```python
from build123d import *

# Parameters (mm, degrees)
SKETCH_1_W          = 18
SKETCH_1_H          = 16
EXTRUDE_1_DEPTH     = 95
CHAMFER_1_SIZE      = 5
CUT_EXTRUDE_1_REACH = 100.005


with BuildPart() as part:
    # 草图1 → 凸台-拉伸1 (new, symmetric)
    with BuildSketch(Plane.XY):
        with Locations((9, 8)):
            Rectangle(SKETCH_1_W, SKETCH_1_H)
    extrude(amount=EXTRUDE_1_DEPTH, both=True)

    # 倒角1
    chamfer_1_edges = [part.edges().sort_by_distance(p)[0] for p in [
        (18, 8, -95),
        (18, 8, 95),
    ]]
    chamfer(chamfer_1_edges, length=CHAMFER_1_SIZE)

    # 草图2 → 切除-拉伸1 (cut, up to next)
    with BuildSketch(Plane.XZ, mode=Mode.PRIVATE) as cut_extrude_1_sk1:
        with BuildLine():
            Line((5.5, 83), (10.5, 83))
            ThreePointArc((10.5, 83), (13, 80.5), (10.5, 78))
            Line((10.5, 78), (5.5, 78))
            ThreePointArc((5.5, 78), (3, 80.5), (5.5, 83))
        make_face()
    cut_extrude_1_tool1 = extrude(cut_extrude_1_sk1.sketch, amount=-CUT_EXTRUDE_1_REACH, mode=Mode.PRIVATE) & part.part
    # 草图2 → 切除-拉伸1 (cut, up to next)
    with BuildSketch(Plane.XZ, mode=Mode.PRIVATE) as cut_extrude_1_sk2:
        with BuildLine():
            Line((5.5, 2.5), (10.5, 2.5))
            ThreePointArc((10.5, 2.5), (13, 0), (10.5, -2.5))
            Line((10.5, -2.5), (5.5, -2.5))
            ThreePointArc((5.5, -2.5), (3, 0), (5.5, 2.5))
        make_face()
    cut_extrude_1_tool2 = extrude(cut_extrude_1_sk2.sketch, amount=-CUT_EXTRUDE_1_REACH, mode=Mode.PRIVATE) & part.part
    # 草图2 → 切除-拉伸1 (cut, up to next)
    with BuildSketch(Plane.XZ, mode=Mode.PRIVATE) as cut_extrude_1_sk3:
        with BuildLine():
            Line((5.5, -83), (10.5, -83))
            ThreePointArc((10.5, -83), (13, -80.5), (10.5, -78))
            Line((10.5, -78), (5.5, -78))
            ThreePointArc((5.5, -78), (3, -80.5), (5.5, -83))
        make_face()
    cut_extrude_1_tool3 = extrude(cut_extrude_1_sk3.sketch, amount=-CUT_EXTRUDE_1_REACH, mode=Mode.PRIVATE) & part.part
    add(cut_extrude_1_tool1.solids().sort_by_distance((8, 0, 80.5))[0], mode=Mode.SUBTRACT)
    add(cut_extrude_1_tool2.solids().sort_by_distance((8, 0, 0))[0], mode=Mode.SUBTRACT)
    add(cut_extrude_1_tool3.solids().sort_by_distance((8, 0, -80.5))[0], mode=Mode.SUBTRACT)


solid = part.part
```
Work out the finished part from the listing and answer in its coordinate system (mm). A direction names the side the tool comes from. Give positions to 0.01 mm unless a question says otherwise; leave off trailing zeros. Order: outer loops, then holes, each group sorted by start corner. A loop starts at its lowest first (then second) coordinate and runs counter-clockwise, first axis right, second up. Notation, with made-up numbers: (68.5, -8) -> (72.5, -8) arc R30 cw to (72.5, 30) -> close; hole circle Ø3 at (62.25, -19.5). An arc over 180 degrees is marked (long way). Answer as CSV lines item,"result". Start each with the question number.
(1) Section A-A, the plane x = 7.25 is taken. Write down the section's boundary in (y, z).
(2) For a pull along X with two mould halves and no side action, classify faces 3 (the cylindrical face through (3, 8, 0)), 4 (the flat face through (8, 8, 2.5)), 5 (the flat face through (18, 8, 1)), 6 (the flat face through (6, 8, -95)) as released by +X, released by -X, zero draft, split by the parting line, or undercut.
(3) Section C-C, the plane z = -80.5 is taken. Write down the section's boundary in (x, y), plus the area to 3 significant figures.
(4) Consider line 1 along Z through (x, y) = (6.75, 12); line 2 along Z through (x, y) = (5, 13.5); line 3 along Z through (x, y) = (16.75, 3). Determine where each line is inside the solid, lowest interval first.
(5) Section B-B, the plane y = 12.5 is taken. Write down the section's boundary in (x, z).
(6) Which of the six approach directions +Z, -Z, +X, -X, +Y, -Y give full straight-line access (tool end or side, diameter ignored) to faces 1 (the flat face through (16, 8, 92)), 2 (the cylindrical face through (3, 7.9, -80.4))?
Entries:
1,outline,"(0, -95) -> (16, -95) -> (16, -83) -> (0, -83) -> close; (0, -78) -> (16, -78) -> (16, -2.5) -> (0, -2.5) -> close; (0, 2.5) -> (16, 2.5) -> (16, 78) -> (0, 78) -> close; (0, 83) -> (16, 83) -> (16, 95) -> (0, 95) -> close"
2,face 3,"undercut"
2,face 4,"undercut"
2,face 5,"released by +X"
2,face 6,"zero draft"
3,outline,"(0, 0) -> (3, 0) -> (3, 16) -> (0, 16) -> close; (13, 0) -> (18, 0) -> (18, 16) -> (13, 16) -> close"
3,area,"128 mm²"
4,line 1,"-95 to -83, -78 to -2.5, 2.5 to 78, 83 to 95"
4,line 2,"-95 to -82.95, -78.05 to -2.45, 2.45 to 78.05, 82.95 to 95"
4,line 3,"-91.25 to 91.25"
5,outline,"(0, -95) -> (13, -95) -> (18, -90) -> (18, 90) -> (13, 95) -> (0, 95) -> close; hole (5.5, -83) -> (10.5, -83) arc R2.5 ccw to (10.5, -78) -> (5.5, -78) arc R2.5 ccw to start; hole (5.5, -2.5) -> (10.5, -2.5) arc R2.5 ccw to (10.5, 2.5) -> (5.5, 2.5) arc R2.5 ccw to start; hole (5.5, 78) -> (10.5, 78) arc R2.5 ccw to (10.5, 83) -> (5.5, 83) arc R2.5 ccw to start"
6,face 1,"+Z, +X, +Y, -Y"
6,face 2,"+Y, -Y"
